Work out the finished part from the listing and answer in its coordinate system (mm). Round coordinates to 2 decimals unless told otherwise and drop trailing zeros. Write each loop counter-clockwise with the first axis right and the second up, starting at its lowest first coordinate (ties: lowest second). Pieces come first, ordered by that corner, then holes.
1. Straight lines are drawn through the part: probe 1 along Y at (x, z) = (-13.5, -0.1); probe 2 along X at (y, z) = (1, -1.1); probe 3 along X at (y, z) = (-0.75, -0.4). For each, find the intervals that lie inside material, in ascending order.
2. Find section C-C (z = 0.8). Write down the section's boundary in (x, y), and give its area (3 significant figures).
3. Determine the mould class of faces 1 (the face through (-11.354, 0.676, -0.021)), 2 (the face through (13.21, 2.23, -0.02)), 3 (the face through (17.5, 0, 0)), 4 (the face through (-17.5, 0, 0)) for opening direction X: pulls with the +X half, pulls with the -X half, needs draft (parallel to the pull), parting line crosses it, or undercut.
4. Find section B-B (x = 13.5). Write down the section's boundary in (y, z).
5. Find section A-A (y = 0). Write down the section's boundary in (x, z).
```python
from build123d import *

# Parameters (mm, degrees)
SKETCH_1_W      = 35
SKETCH_1_H      = 9
SKETCH_1_R      = 2.25
EXTRUDE_1_DEPTH = 1.5


with BuildPart() as part:
    # 草图1 → 凸台-拉伸1 (new, symmetric)
    with BuildSketch(Plane.XY):
        Rectangle(SKETCH_1_W, SKETCH_1_H)
        with Locations((-13.5, 0)):
            Circle(SKETCH_1_R, mode=Mode.SUBTRACT)
        with Locations((13.5, 0)):
            Circle(SKETCH_1_R, mode=Mode.SUBTRACT)
    extrude(amount=EXTRUDE_1_DEPTH, both=True)


solid = part.part
```
Worked answers:
1. probe 1: y = -4.5 to -2.25, 2.25 to 4.5
1. probe 2: x = -17.5 to -15.52, -11.48 to 11.48, 15.52 to 17.5
1. probe 3: x = -17.5 to -15.62, -11.38 to 11.38, 15.62 to 17.5
2. outline: (-17.5, -4.5) - (17.5, -4.5) - (17.5, 4.5) - (-17.5, 4.5) - close; hole circle Ø4.5 at (-13.5, 0); hole circle Ø4.5 at (13.5, 0)
2. area: 283 mm2
3. face 1: undercut
3. face 2: undercut
3. face 3: pulls with the +X half
3. face 4: pulls with the -X half
4. outline: (-4.5, -1.5) - (-2.25, -1.5) - (-2.25, 1.5) - (-4.5, 1.5) - close; (2.25, -1.5) - (4.5, -1.5) - (4.5, 1.5) - (2.25, 1.5) - close
5. outline: (-17.5, -1.5) - (-15.75, -1.5) - (-15.75, 1.5) - (-17.5, 1.5) - close; (-11.25, -1.5) - (11.25, -1.5) - (11.25, 1.5) - (-11.25, 1.5) - close; (15.75, -1.5) - (17.5, -1.5) - (17.5, 1.5) - (15.75, 1.5) - close
